```python
from build123d import *

# Parameters (mm, degrees)
SKETCH1_R           = 50
BOSS_EXTRUDE1_DEPTH = 8
SKETCH2_R           = 2.5
CUT_EXTRUDE1_DEPTH  = 8
SKETCH3_R           = 2.1
CUT_EXTRUDE2_DEPTH  = 8
SKETCH4_R           = 4
CUT_EXTRUDE3_DEPTH  = 4
SKETCH5_R           = 2.5
CUT_EXTRUDE4_DEPTH  = 4
SKETCH6_R           = 35
CUT_EXTRUDE5_DEPTH  = 10


with BuildPart() as part:
    # Sketch1 → Boss-Extrude1 (new body)
    with BuildSketch(Plane.XY):
        Circle(SKETCH1_R)
    extrude(amount=BOSS_EXTRUDE1_DEPTH)

    # Sketch2 → Cut-Extrude1 (cut)
    with BuildSketch(Plane.XY.offset(8)):
        with Locations((-30.054076263, 30.05)):
            Circle(SKETCH2_R)
        with Locations((30.054076263, 30.05)):
            Circle(SKETCH2_R)
        with Locations((-30.054076263, -30.05)):
            Circle(SKETCH2_R)
        with Locations((30.054076263, -30.05)):
            Circle(SKETCH2_R)
    extrude(amount=-CUT_EXTRUDE1_DEPTH, mode=Mode.SUBTRACT)

    # Sketch3 → Cut-Extrude2 (cut)
    with BuildSketch(Plane.XY.offset(8)):
        with Locations((0, 42.5)):
            Circle(SKETCH3_R)
    extrude(amount=-CUT_EXTRUDE2_DEPTH, mode=Mode.SUBTRACT)

    # Sketch4 → Cut-Extrude3 (cut)
    with BuildSketch(Plane.XY.offset(8)):
        with Locations((0, -42.5)):
            Circle(SKETCH4_R)
        with Locations((-36.806079661, 21.25)):
            Circle(SKETCH4_R)
        with Locations((36.806079661, 21.25)):
            Circle(SKETCH4_R)
    extrude(amount=-CUT_EXTRUDE3_DEPTH, mode=Mode.SUBTRACT)

    # Sketch5 → Cut-Extrude4 (cut)
    with BuildSketch(Plane.XY.offset(4)):
        with Locations((-36.806079661, 21.25)):
            Circle(SKETCH5_R)
        with Locations((0, -42.5)):
            Circle(SKETCH5_R)
        with Locations((36.806079661, 21.25)):
            Circle(SKETCH5_R)
    extrude(amount=-CUT_EXTRUDE4_DEPTH, mode=Mode.SUBTRACT)

    # Sketch6 → Cut-Extrude5 (cut)
    with BuildSketch(Plane.XY.offset(8)):
        Circle(SKETCH6_R)
    extrude(amount=-CUT_EXTRUDE5_DEPTH, mode=Mode.SUBTRACT)


solid = part.part
```
Geometry check sheet. Reference: the model listing, model coordinates, mm. A direction names the side the tool comes from. Coordinates: 2 decimals unless noted, no trailing zeros. Write each loop counter-clockwise with the first axis right and the second up, starting at its lowest first coordinate (ties: lowest second). Pieces come first, ordered by that corner, then holes. Notation, with made-up numbers: M 33.25,43 L 51.25,43 A15 ccw 51.25,56 Z; hole C 66.5,74.25 d9. An arc over 180 degrees is marked long. Use one line per item in the form item = value. Start each with the question number.
1) Section check D-D on y = 21.25. Enter the section's corners in (x, z), and give its area (3 significant figures).
2) Release check for a two-part mould opening along X. For faces 1 (the flat face through (10, 34, 0)), 2 (the cylindrical face through (47.69, 15.02, 3.94)), 3 (the cylindrical face through (-27.745, -31.008, 4.056)) record: pulls with the +X half, pulls with the -X half, needs draft (parallel to the pull), parting line crosses it, or undercut.
3) Section check C-C on x = 22.5. Enter the section's corners in (y, z), and give its area (3 significant figures).
4) Thickness scan on probe 1 along Y at (x, z) = (1, 6.5); probe 2 along X at (y, z) = (-32, 4); probe 3 along Y at (x, z) = (-12, 3.75). Record the ranges inside material, lowest first. Write a range as from..to.
5) Go/stop test with flat-tipped pins: pin 1 Ø6.5 at (x, y) = (-36.81, 21.25) entering from +Z; pin 2 Ø1.5 at (y, z) = (1, 4.5) entering from +X; pin 3 Ø1.5 at (y, z) = (-18, 6) entering from +X; pin 4 Ø4 at (x, y) = (-36.81, 21.25) entering from -Z. Record where each tip stops, or that it passes through.
6) Section check B-B on z = 6. State how many separate pieces and enclosed holes the cut face has, and give its area (3 significant figures).
7) Set-up check for faces 4 (the cylindrical face through (-28.9, 27.832, 4.056)), 5 (the flat face through (-34, 21, 4)): record each of +Z, -Z, +X, -X, +Y, -Y from which the full face is reachable in a straight line by a thin tool's end or side.
8) Section check A-A on y = 0. Enter the section's corners in (x, z).
Responses:
q1.outline = M -45.26,0 L -39.31,0 L -39.31,4 L -40.81,4 L -40.81,8 L -45.26,8 Z; M -34.31,0 L -27.81,0 L -27.81,8 L -32.81,8 L -32.81,4 L -34.31,4 Z; M 27.81,0 L 34.31,0 L 34.31,4 L 32.81,4 L 32.81,8 L 27.81,8 Z; M 39.31,0 L 45.26,0 L 45.26,8 L 40.81,8 L 40.81,4 L 39.31,4 Z
q1.area = 175 mm2
q2.face_1 = needs draft
q2.face_2 = parting line crosses it
q2.face_3 = undercut
q3.outline = M -44.65,0 L -26.81,0 L -26.81,8 L -44.65,8 Z; M 26.81,0 L 44.65,0 L 44.65,8 L 26.81,8 Z
q3.area = 285 mm2
q4.probe_1 = -49.99..-46.37, -38.63..-34.99, 34.99..40.65, 44.35..49.99
q4.probe_2 = -38.42..-31.62, -28.49..-14.18, 14.18..28.49, 31.62..38.42
q4.probe_3 = -48.54..-32.88, 32.88..48.54
q5.pin_1 = 4
q5.pin_2 = 50
q5.pin_3 = 46.93
q5.pin_4 = through
q6.separate_pieces = 1
q6.enclosed_holes = 9
q6.area = 3,760 mm2
q7.face_4 = +Z, -Z
q7.face_5 = +Z
q8.outline = M -50,0 L -35,0 L -35,8 L -50,8 Z; M 35,0 L 50,0 L 50,8 L 35,8 Z
